CAD build for the part. Positions are in the model's coordinates, mm. Face numbers are marked on the shaded views. A direction names the side the tool comes from. Round coordinates to 2 decimals unless told otherwise and drop trailing zeros. Loops run counter-clockwise (first coordinate to the right, second up) from the corner with the lowest first, then second, coordinate; pieces in that order, holes last. Notation, with made-up numbers: (42, 27.25) - (72, 27.25) arc R29 cw to (72, 62.25) - close; hole circle Ø8 at (-39.75, 46). An arc over 180 degrees is marked (long way). One line per question, with ' | ' between items.
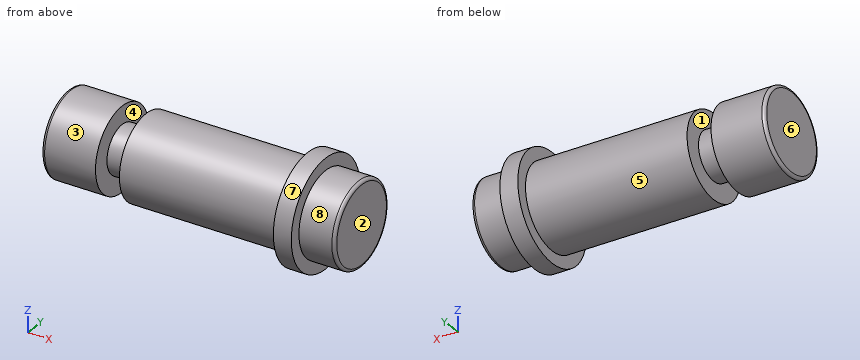
```python
from build123d import *

# Parameters (mm, degrees)
FILLET1_R = 0.5


with BuildPart() as part:
    # Sketch1 → Revolve1 (revolve)
    with BuildSketch(Plane.XY, mode=Mode.PRIVATE) as revolve1_sk:
        Polygon((0, 0), (0, 7), (9, 7), (9, 4), (13, 4), (13, 7), (40, 7), (40, 9), (43, 9), (43, 7), (49, 7), (49, 0), align=None)
    revolve(revolve1_sk.sketch.rotate(Axis((49, 0, 0), (-1, 0, 0)), 90), axis=Axis((49, 0, 0), (-1, 0, 0)))

    # Fillet1
    fillet1_edges = [part.edges().sort_by_distance(p)[0] for p in [
        (0, 0, 7),
        (49, 0, 7),
    ]]
    fillet(fillet1_edges, radius=FILLET1_R)


solid = part.part
```
(1) Probe L1, parallel to X at y = -2.5, z = 6; L2, parallel to X at y = -0.5, z = -7.5; L3, parallel to X at y = 6.75, z = -1.5. List the from-to ranges inside material, lowest first.
Results found:
L1: x = 0 to 9, 13 to 49 | L2: x = 40 to 43 | L3: x = 0.22 to 9, 13 to 48.78
(2) Tool access for the marked faces 4, 5, 6, 7 and 8: list every direction of +Z, -Z, +X, -X, +Y, -Y with a clear straight run to the whole face (end or side of a thin tool).
Results found:
face 4: none | face 5: -X | face 6: +Z, -Z, -X, +Y, -Y | face 7: +X, -X | face 8: +X
(3) Two-plate mould, pull along X, no slides. Class the marked faces 1, 2 and 3: released by +X, released by -X, zero draft, split by the parting line, or undercut.
Results found:
face 1: undercut | face 2: released by +X | face 3: zero draft
(4) Drop flat-ended pins along their axis: P1, Ø6, axis at x = 32.5, y = 1.5, coming from the -Z side; P2, Ø1, axis at x = 39, y = 4, coming from the -Z side; P3, Ø2, axis at x = 7.5, z = -3.5, coming from the -Y side. Give the stop position or say it passes through.
Results found:
P1: stops at z = -7 | P2: stops at z = -6.06 | P3: stops at y = -6.54
(5) Cut at C-C, the plane x = 28. Write the cut outline in (y, z).
Results found:
outline: circle Ø14 at (0, 0)
(6) Cut at A-A, the plane y = 0. Write the cut outline in (x, z).
Results found:
outline: (0, -6.5) arc R0.5 ccw to (0.5, -7) - (9, -7) - (9, -4) - (13, -4) - (13, -7) - (40, -7) - (40, -9) - (43, -9) - (43, -7) - (48.5, -7) arc R0.5 ccw to (49, -6.5) - (49, 6.5) arc R0.5 ccw to (48.5, 7) - (43, 7) - (43, 9) - (40, 9) - (40, 7) - (13, 7) - (13, 4) - (9, 4) - (9, 7) - (0.5, 7) arc R0.5 ccw to (0, 6.5) - close
